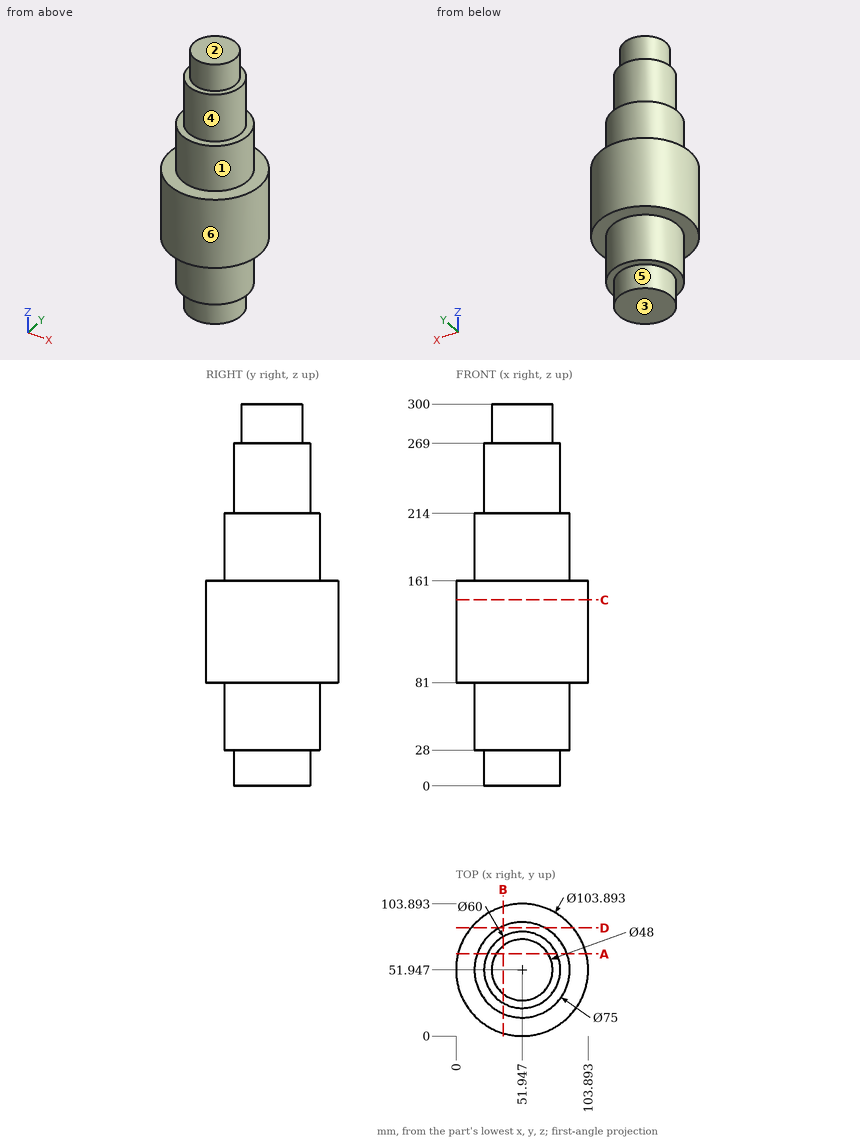
Job drawing, mm, ordinate dimensions from the low corner. One solid piece. A direction names the side the tool comes from. Coordinates: 2 decimals unless noted, no trailing zeros. Order: outer loops, then holes, each group sorted by start corner. A loop starts at its lowest first (then second) coordinate and runs counter-clockwise, first axis right, second up. Notation, with made-up numbers: (-32, 79.25) -> (8, 79.25) arc R20 cw to (8, 92.25) -> close; hole circle Ø10 at (-20.75, 43.25). An arc over 180 degrees is marked (long way). Put each result on its own line as item: value. Start each with the question number.
(1) Band-saw the part on B-B (x = 37). Give the cut face in (y, z) (1 decimal).
(2) Pin check, flat tips, straight feed: pin 1 Ø6 at (x, z) = (42, 215) entering from -Y; pin 2 Ø1.5 at (x, z) = (67, 216.5) entering from -Y (1 decimal); pin 3 Ø1.5 at (x, z) = (78.5, 260.5) entering from -Y (1 decimal). Stop position of each tip, or through.
(3) Mould opens along Z. For the marked faces 1, 2 and 3 say: pulls with the +Z half, pulls with the -Z half, needs draft (parallel to the pull), parting line crosses it, or undercut.
(4) Which spindle directions (+Z, -Z, +X, -X, +Y, -Y) get a long thin tool onto all of the face, cutting with end or side? Do the marked faces 4, 5 and 6. Say none if no direction does.
(5) Band-saw the part on A-A (y = 64.5). Give the cut face in (x, z), then the cut area to 3 significant figures.
(6) Probe line 1 along Z through (x, y) = (21, 49); line 2 along X through (y, z) = (54, 167.5); line 3 along Z through (x, y) = (95.5, 52). List the from-to ranges inside material, lowest first. Write a range as [from, to].
(7) Band-saw the part on C-C (z = 146). Give the cut face in (x, y), then the cut area to 3 significant figures.
(8) Band-saw the part on D-D (y = 85). Give the cut face in (x, z) (1 decimal), then the cut area to 3 significant figures.
Determined:
1. outline: (2.2, 81) -> (17.6, 81) -> (17.6, 28) -> (25.9, 28) -> (25.9, 0) -> (78, 0) -> (78, 28) -> (86.3, 28) -> (86.3, 81) -> (101.7, 81) -> (101.7, 161) -> (86.3, 161) -> (86.3, 214) -> (78, 214) -> (78, 269) -> (70.7, 269) -> (70.7, 300) -> (33.2, 300) -> (33.2, 269) -> (25.9, 269) -> (25.9, 214) -> (17.6, 214) -> (17.6, 161) -> (2.2, 161) -> close
2. pin 1: stops at y = 15.13
2. pin 2: stops at y = 25.6
2. pin 3: stops at y = 36.6
3. face 1: needs draft
3. face 2: pulls with the +Z half
3. face 3: pulls with the -Z half
4. face 4: +Z
4. face 5: -Z
4. face 6: +Z, -Z
5. outline: (1.54, 81) -> (16.61, 81) -> (16.61, 28) -> (24.7, 28) -> (24.7, 0) -> (79.19, 0) -> (79.19, 28) -> (87.28, 28) -> (87.28, 81) -> (102.35, 81) -> (102.35, 161) -> (87.28, 161) -> (87.28, 214) -> (79.19, 214) -> (79.19, 269) -> (72.4, 269) -> (72.4, 300) -> (31.49, 300) -> (31.49, 269) -> (24.7, 269) -> (24.7, 214) -> (16.61, 214) -> (16.61, 161) -> (1.54, 161) -> close
5. area: 21,300 mm²
6. line 1: z = [28, 214]
6. line 2: x = [14.5, 89.39]
6. line 3: z = [81, 161]
7. outline: circle Ø103.89 at (51.95, 51.95)
7. area: 8,480 mm²
8. outline: (11.9, 81) -> (34.2, 81) -> (34.2, 28) -> (69.7, 28) -> (69.7, 81) -> (92, 81) -> (92, 161) -> (69.7, 161) -> (69.7, 214) -> (34.2, 214) -> (34.2, 161) -> (11.9, 161) -> close
8. area: 10,200 mm²
